Study the drawing (mm; zero at the part's minimum x, y, z) and answer. Round coordinates to 2 decimals unless told otherwise and drop trailing zeros. Write each loop counter-clockwise with the first axis right and the second up, starting at its lowest first coordinate (ties: lowest second). Pieces come first, ordered by that corner, then holes. Notation, with made-up numbers: (23, -18.75) - (50, -18.75) arc R14 ccw to (50, -9.75) - close; hole circle Ø3 at (-16, -5.5). An arc over 180 degrees is marked (long way). Use one line per item in the form item = value. Start each with the question number.
1) For a pull along Y with two mould halves and no side action, classify the marked faces 1, 2, 3 and 4 as released by +Y, released by -Y, zero draft, split by the parting line, or undercut.
2) The part is cut by section B-B, the plane z = 1.5. Give the vertices of the cut face in (x, y).
3) The part is cut by section A-A, the plane x = 35. Give the vertices of the cut face in (y, z), plus the area to 3 significant figures.
4) Consider line 1 along X through (y, z) = (48, 6); line 2 along Y through (x, z) = (35, 6); line 3 along Y through (x, z) = (78, 2). Determine where each line is inside the solid, lowest interval first. Write a range as from..to.
5) The part is cut by section C-C, the plane y = 50. Give the vertices of the cut face in (x, z), plus the area to 3 significant figures.
6) The part is cut by section D-D, the plane x = 78. Give the vertices of the cut face in (y, z).
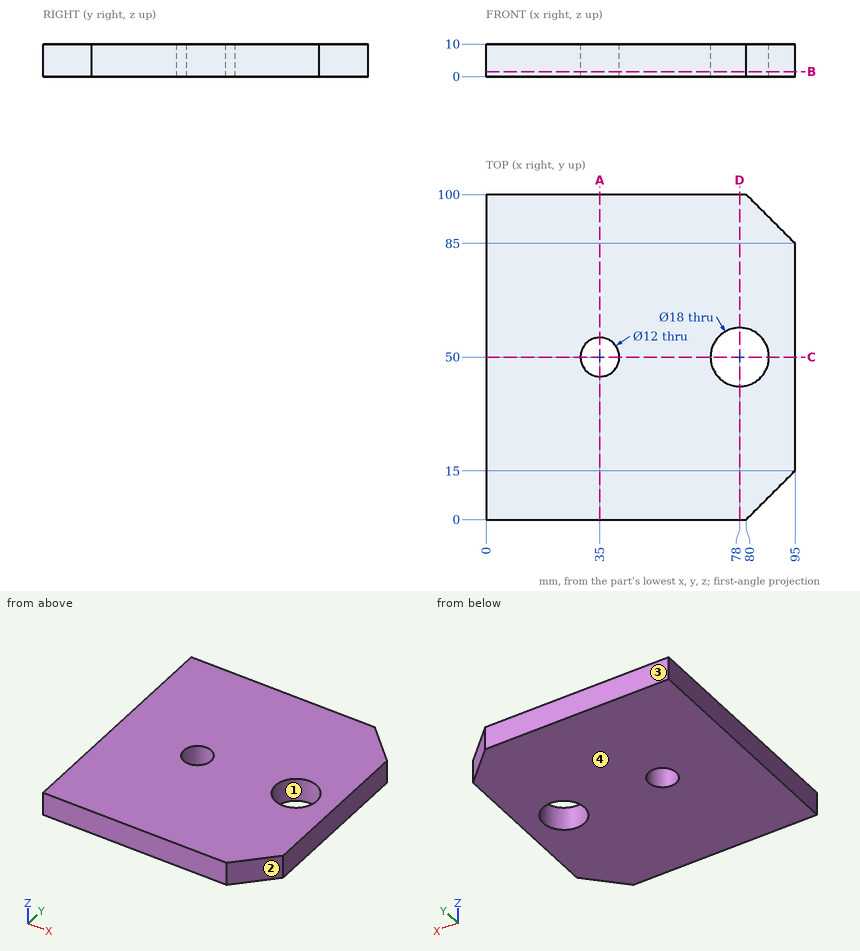
Geometry results:
q1.face_1 = undercut
q1.face_2 = released by -Y
q1.face_3 = released by +Y
q1.face_4 = zero draft
q2.outline = (0, 0) - (80, 0) - (95, 15) - (95, 85) - (80, 100) - (0, 100) - close; hole circle Ø12 at (35, 50); hole circle Ø18 at (78, 50)
q3.outline = (0, 0) - (44, 0) - (44, 10) - (0, 10) - close; (56, 0) - (100, 0) - (100, 10) - (56, 10) - close
q3.area = 880 mm2
q4.line_1 = 0..29.34, 40.66..69.23, 86.77..95
q4.line_2 = 0..44, 56..100
q4.line_3 = 0..41, 59..100
q5.outline = (0, 0) - (29, 0) - (29, 10) - (0, 10) - close; (41, 0) - (69, 0) - (69, 10) - (41, 10) - close; (87, 0) - (95, 0) - (95, 10) - (87, 10) - close
q5.area = 650 mm2
q6.outline = (0, 0) - (41, 0) - (41, 10) - (0, 10) - close; (59, 0) - (100, 0) - (100, 10) - (59, 10) - close
